from build123d import *

# Parameters (mm, degrees)
SKETCH_1_W          = 14
SKETCH_1_H          = 185
EXTRUDE_1_DEPTH     = 150
SKETCH_2_W          = 300
SKETCH_2_H          = 20
SKETCH_2_H_2        = 21
CUT_EXTRUDE_1_DEPTH = 1.5
CUT_EXTRUDE_2_REACH = 240.581
SKETCH_3_W          = 174
SKETCH_3_H          = 56
FILLET_1_R          = 5


with BuildPart() as part:
    # 草图1 → 凸台-拉伸1 (new, symmetric)
    with BuildSketch(Plane.XY):
        with Locations((7, 92.5)):
            Rectangle(SKETCH_1_W, SKETCH_1_H)
    extrude(amount=EXTRUDE_1_DEPTH, both=True)

    # 草图2 → 切除-拉伸1 (cut)
    with BuildSketch(Plane(origin=(14, 0, 0), x_dir=(0, 0, -1), z_dir=(1, 0, 0))):
        with Locations((0, 175)):
            Rectangle(SKETCH_2_W, SKETCH_2_H)
        with Locations((0, 69.5)):
            Rectangle(SKETCH_2_W, SKETCH_2_H_2)
    extrude(amount=-CUT_EXTRUDE_1_DEPTH, mode=Mode.SUBTRACT)

    # 草图3 → 切除-拉伸2 (cut, up to next)
    with BuildSketch(Plane(origin=(14, 0, 0), x_dir=(0, 0, -1), z_dir=(1, 0, 0)), mode=Mode.PRIVATE) as cut_extrude_2_sk1:
        with Locations((0, 122.5)):
            Rectangle(SKETCH_3_W, SKETCH_3_H)
    cut_extrude_2_tool1 = extrude(cut_extrude_2_sk1.sketch, amount=-CUT_EXTRUDE_2_REACH, mode=Mode.PRIVATE) & part.part
    add(cut_extrude_2_tool1.solids().sort_by_distance((14, 122.5, 0))[0], mode=Mode.SUBTRACT)

    # 圆角1
    fillet_1_edges = [part.edges().sort_by_distance(p)[0] for p in [
        (7, 150.5, -87),
        (7, 94.5, -87),
        (7, 94.5, 87),
        (7, 150.5, 87),
    ]]
    fillet(fillet_1_edges, radius=FILLET_1_R)


solid = part.part
Build history of the part. All positions in model axes, mm. A direction names the side the tool comes from. Give positions to 0.01 mm unless a question says otherwise; leave off trailing zeros. Loops run counter-clockwise (first coordinate to the right, second up) from the corner with the lowest first, then second, coordinate; pieces in that order, holes last. Notation, with made-up numbers: (49.5, 89.25) - (63.5, 89.25) arc R19 ccw to (63.5, 116.25) - close; hole circle Ø7 at (9.5, 62). An arc over 180 degrees is marked (long way). Write item = value, one per line. Start each with the question number.
1) Probe probe 1 along Z at (x, y) = (11.25, 136.5); probe 2 along Y at (x, z) = (1, 78); probe 3 along X at (y, z) = (61, -59.5). List the from-to ranges inside material, lowest first. Write a range as from..to.
2) Drop flat-ended pins along their axis: pin 1 Ø6.5 at (y, z) = (73.5, 12) entering from +X; pin 2 Ø1.2 at (x, z) = (13.5, 53.5) entering from -Y; pin 3 Ø0.8 at (x, z) = (13, 19) entering from +Y. Give the stop position or say it passes through.
3) Band-saw the part on C-C on x = 6.75. Give the cut face in (y, z), plus the area to 3 significant figures.
4) Band-saw the part on D-D on z = 92.5. Give the cut face in (x, y), plus the area to 3 significant figures.
5) Band-saw the part on A-A on z = -42.5. Give the cut face in (x, y).
6) Pull direction Y, two halves, no side cores. Call faces 5 (the flat face through (7, 0, 2)), 6 (the flat face through (14, 29, 2)), 7 (the flat face through (7, 122, -87)): +Y half, -Y half, draft (parallel to the pull), parting line (faces both ways), or undercut.
7) Tool access for faces 1 (the flat face through (14, 94, 2)), 2 (the flat face through (7, 150.5, 1)), 3 (the flat face through (12.5, 70, 2)), 4 (the flat face through (12.5, 175, 2)): list every direction of +Z, -Z, +X, -X, +Y, -Y with a clear straight run to the whole face (end or side of a thin tool).
8) Band-saw the part on B-B on y = 141.5. Give the cut face in (x, z), plus the area to 3 significant figures.
Final values:
q1.probe_1 = -150..-87, 87..150
q1.probe_2 = 0..94.5, 150.5..185
q1.probe_3 = 0..12.5
q2.pin_1 = 12.5
q2.pin_2 = 0
q2.pin_3 = 165
q3.outline = (0, -150) - (185, -150) - (185, 150) - (0, 150) - close; hole (94.5, -82) arc R5 ccw to (99.5, -87) - (145.5, -87) arc R5 ccw to (150.5, -82) - (150.5, 82) arc R5 ccw to (145.5, 87) - (99.5, 87) arc R5 ccw to (94.5, 82) - close
q3.area = 45,800 mm²
q4.outline = (0, 0) - (14, 0) - (14, 59) - (12.5, 59) - (12.5, 80) - (14, 80) - (14, 165) - (12.5, 165) - (12.5, 185) - (0, 185) - close
q4.area = 2,530 mm²
q5.outline = (0, 0) - (14, 0) - (14, 59) - (12.5, 59) - (12.5, 80) - (14, 80) - (14, 94.5) - (0, 94.5) - close; (0, 150.5) - (14, 150.5) - (14, 165) - (12.5, 165) - (12.5, 185) - (0, 185) - close
q6.face_5 = -Y half
q6.face_6 = draft
q6.face_7 = undercut
q7.face_1 = +Z, -Z, +X, +Y, -Y
q7.face_2 = +X, -X
q7.face_3 = +Z, -Z, +X
q7.face_4 = +Z, -Z, +X, +Y
q8.outline = (0, -150) - (14, -150) - (14, -87) - (0, -87) - close; (0, 87) - (14, 87) - (14, 150) - (0, 150) - close
q8.area = 1,760 mm²
